Geometry: see drawing. Coordinates: mm, zero at the bounding-box minimum. A direction names the side the tool comes from. Round coordinates to 2 decimals unless told otherwise and drop trailing zeros. Write each loop counter-clockwise with the first axis right and the second up, starting at its lowest first coordinate (ties: lowest second). Pieces come first, ordered by that corner, then holes. Notation, with made-up numbers: (47.25, 17) - (84.25, 17) arc R12 cw to (84.25, 37) - close; hole circle Ø11 at (9, 3). An arc over 180 degrees is marked (long way). One line per item, written item: value. Start each with the question number.
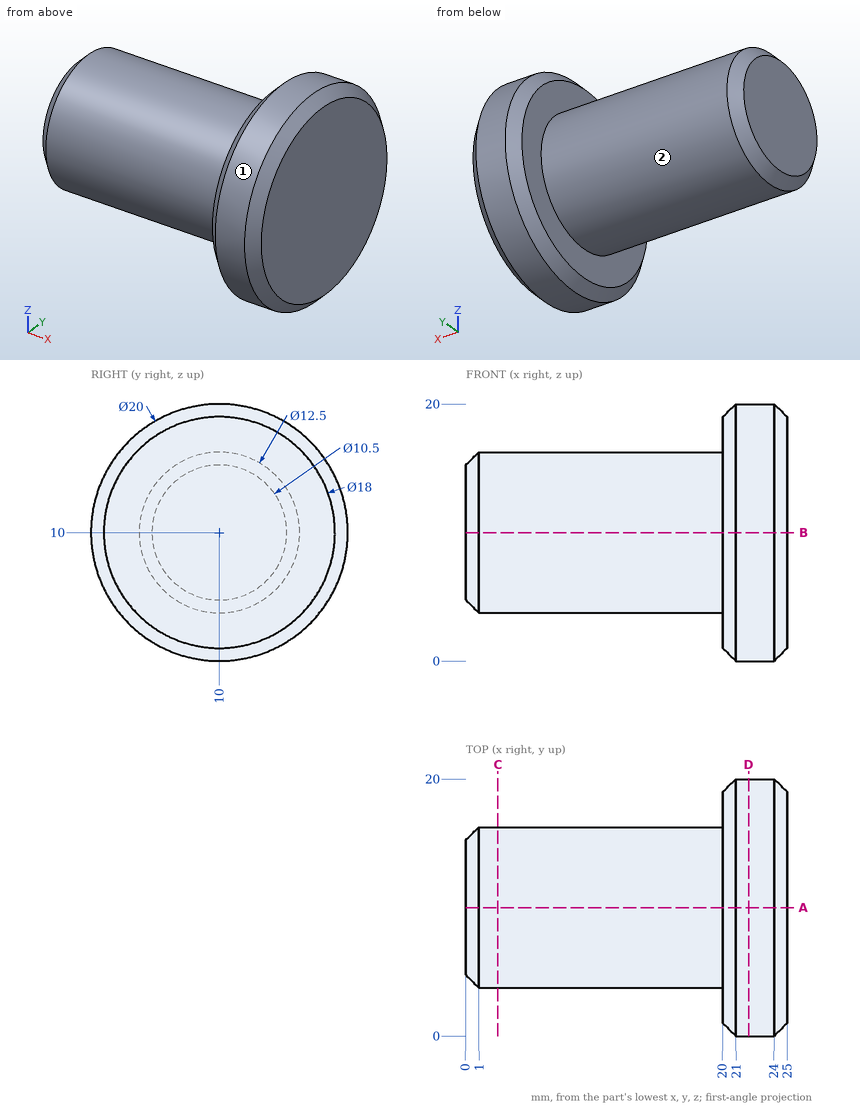
Q1. Cut plane A-A, the plane y = 10. Output: boundary loops of the cut face in (x, z), and give its area (3 significant figures).
Q2. Material intervals for probe 1 along X at (y, z) = (7.25, 16); probe 2 along Y at (x, z) = (15.75, 10); probe 3 along Z at (x, y) = (14.75, 6.5), sorted ascending. Write a range as from..to.
Q3. Access query for the marked faces 1 and 2. Directions: +Z, -Z, +X, -X, +Y, -Y. A direction counts if a zero-diameter tool reaches every point of the face in a straight line with its end or side. Return the directions, or none.
Q4. Contact query for flat-ended pins moving along their axis: pin 1 Ø1 at (x, y) = (9, 8) entering from +Z; pin 2 Ø1 at (x, z) = (8, 7.5) entering from +Y; pin 3 Ø12 at (x, z) = (11.5, 11.5) entering from +Y. Output: stop coordinate, or through.
Q5. Cut plane D-D, the plane x = 22. Output: boundary loops of the cut face in (y, z).
Q6. Cut plane C-C, the plane x = 2.5. Output: boundary loops of the cut face in (y, z).
A:
1. outline: (0, 4.75) - (1, 3.75) - (20, 3.75) - (20, 1) - (21, 0) - (24, 0) - (25, 1) - (25, 19) - (24, 20) - (21, 20) - (20, 19) - (20, 16.25) - (1, 16.25) - (0, 15.25) - close
1. area: 347 mm²
2. probe 1: x = 20..25
2. probe 2: y = 3.75..16.25
2. probe 3: z = 4.82..15.18
3. face 1: +X, -X
3. face 2: -X
4. pin 1: stops at z = 16.07
4. pin 2: stops at y = 15.92
4. pin 3: stops at y = 16.25
5. outline: circle Ø20 at (10, 10)
6. outline: circle Ø12.5 at (10, 10)
